```python
from build123d import *

# Parameters (mm, degrees)
SKETCH_1_R      = 6
EXTRUDE_1_DEPTH = 20


with BuildPart() as part:
    # 草图1 → 凸台-拉伸1 (new, symmetric)
    with BuildSketch(Plane.XY):
        Circle(SKETCH_1_R)
    extrude(amount=EXTRUDE_1_DEPTH, both=True)

    # 草图3 → M6 螺纹孔1 (revolve, cut)
    with BuildSketch(Plane(origin=(0, 0, 20), x_dir=(0, -1, 0), z_dir=(1, 0, 0))):
        Polygon((0, 0), (0, 10.502151548), (2.5, 9), (2.5, 0.525), (3.025, 0), align=None)
    hole_wizard_m6_1 = revolve(axis=Axis((0, 0, 26.35), (0, 0, -1)), mode=Mode.SUBTRACT)

    # 镜向1: M6 螺纹孔1 across plane
    add(hole_wizard_m6_1.mirror(Plane.XY), mode=Mode.SUBTRACT)


solid = part.part
```
Could you check a few things on this model? Use its own coordinates, in mm. A direction names the side the tool comes from. Give positions to 0.01 mm unless a question says otherwise; leave off trailing zeros. Order: outer loops, then holes, each group sorted by start corner. A loop starts at its lowest first (then second) coordinate and runs counter-clockwise, first axis right, second up.
Q1. I'm going to push flat-ended pins straight in: P1, Ø1, axis at y = -4.5, z = -11, coming from the -X side; P2, Ø5, axis at x = 2, z = 14, coming from the +Y side; P3, Ø1, axis at x = 2, z = -6, coming from the +Y side; P4, Ø4, axis at y = -3.5, z = -10, coming from the -X side. Where does each tip first touch, or does it pass through?
Q2. For faces 5 (the cylindrical face through (2.44, 0.54, 15.3)), 6 (the cylindrical face through (2.44, 0.54, -15.3)), 7 (the flat face through (3, -3, -20)), which set-ups out of +Z, -Z, +X, -X, +Y, -Y let a thin tool reach every point of the face, with its end or its side?
Q3. Suppose I cut it at C-C, the plane x = 4. Write out the boundary of the cut face in (y, z).
Q4. We'd pull the mould along Y, two halves only. Please class faces 1 (the flat face through (3, -3, 20)), 2 (the conical face through (0.424, 0.094, -9.759)), 3 (the conical face through (0.424, 0.094, 9.759)), 4 (the cylindrical face through (-6, 0, 0)): +Y half, -Y half, draft (parallel to the pull), parting line (faces both ways), or undercut.
Q5. If I drill on line 1 along Y through (x, z) = (0, -14.25); line 2 along X through (y, z) = (-1.5, -11.5); line 3 along Y through (x, z) = (3.25, 6), over which ranges is the centre line in solid material (lowest first)?
Q6. Suppose I cut it at B-B, the plane z = -8. Write out the boundary of the cut face in (x, y).
Q7. Suppose I cut it at A-A, the plane z = 14. Write out the boundary of the cut face in (x, y), and give its area (3 significant figures).
Q8. Suppose I cut it at D-D, the plane y = -4.5. Write out the boundary of the cut face in (x, z).
Solution:
1. P1: stops at x = -4.47
1. P2: stops at y = 6
1. P3: stops at y = 5.81
1. P4: stops at x = -5.81
2. face 5: +Z
2. face 6: -Z
2. face 7: -Z, +X, -X, +Y, -Y
3. outline: (-4.47, -20) - (4.47, -20) - (4.47, 20) - (-4.47, 20) - close
4. face 1: draft
4. face 2: undercut
4. face 3: undercut
4. face 4: parting line
5. line 1: y = -6 to -2.5, 2.5 to 6
5. line 2: x = -5.81 to -2, 2 to 5.81
5. line 3: y = -5.04 to 5.04
6. outline: circle Ø12 at (0, 0)
7. outline: circle Ø12 at (0, 0); hole circle Ø5 at (0, 0)
7. area: 93.5 mm2
8. outline: (-3.97, -20) - (3.97, -20) - (3.97, 20) - (-3.97, 20) - close
